Geometry: see drawing. Coordinates: mm, zero at the bounding-box minimum. A direction names the side the tool comes from. Give positions to 0.01 mm unless a question says otherwise; leave off trailing zeros. Write each loop counter-clockwise with the first axis right and the second up, starting at its lowest first coordinate (ties: lowest second). Pieces come first, ordered by that corner, then holes. Notation, with made-up numbers: (41.25, 77) -> (64.25, 77) arc R6 cw to (64.25, 84) -> close; hole circle Ø10 at (-22, -2). An arc over 180 degrees is marked (long way). Use one line per item in the form item = value. Start each with the question number.
(1) Cut plane D-D, the plane z = 40.5. Output: boundary loops of the cut face in (x, y).
(2) Cut plane A-A, the plane y = 29.2. Output: boundary loops of the cut face in (x, z), and give its area (3 significant figures).
(3) Cut plane C-C, the plane y = 9.2. Output: boundary loops of the cut face in (x, z).
(4) First-contact query: P1, Ø8, axis at y = 17.5, z = 39.5, coming from the +X side; P2, Ø5, axis at x = 21, z = 29, coming from the +Y side; P3, Ø6.5, axis at x = 6, y = 29.2, coming from the -Z side; P4, Ø4, axis at x = 6, y = 9.2, coming from the -Z side. Flat tips, straight axial feed; report the tip coordinate or a pass-through.
(5) Set-up query: the marked faces 1, 2 and 3. Return all of +Z, -Z, +X, -X, +Y, -Y with unobstructed straight access to the full face (end or side cutting, diameter ignored); none if empty.
(6) Cut plane B-B, the plane x = 6. Output: boundary loops of the cut face in (y, z), and give its area (4 significant figures).
(7) Draft query along Z for the marked faces 4, 5 and 6. Return one class per face: pulls with the +Z half, pulls with the -Z half, needs draft (parallel to the pull), parting line crosses it, or undercut.
(8) Material intervals for line 1 along X through (y, z) = (9, 70); line 2 along Y through (x, z) = (6, 70.5); line 3 along X through (y, z) = (7, 8), sorted ascending. Write a range as from..to.
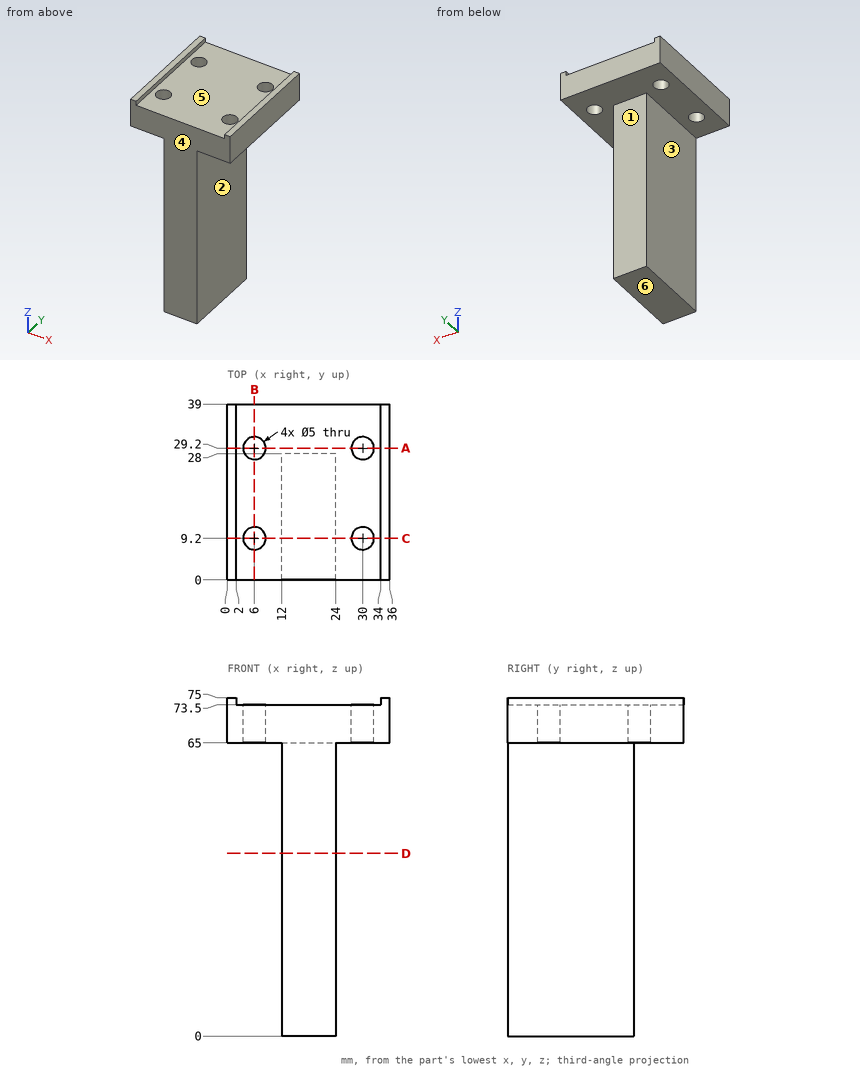
Geometry says:
q1.outline = (12, 0) -> (24, 0) -> (24, 28) -> (12, 28) -> close
q2.outline = (0, 65) -> (3.5, 65) -> (3.5, 73.5) -> (2, 73.5) -> (2, 75) -> (0, 75) -> close; (8.5, 65) -> (27.5, 65) -> (27.5, 73.5) -> (8.5, 73.5) -> close; (32.5, 65) -> (36, 65) -> (36, 75) -> (34, 75) -> (34, 73.5) -> (32.5, 73.5) -> close
q2.area = 227 mm^2
q3.outline = (0, 65) -> (3.5, 65) -> (3.5, 73.5) -> (2, 73.5) -> (2, 75) -> (0, 75) -> close; (8.5, 65) -> (12, 65) -> (12, 0) -> (24, 0) -> (24, 65) -> (27.5, 65) -> (27.5, 73.5) -> (8.5, 73.5) -> close; (32.5, 65) -> (36, 65) -> (36, 75) -> (34, 75) -> (34, 73.5) -> (32.5, 73.5) -> close
q4.P1 = 24
q4.P2 = 28
q4.P3 = 65
q4.P4 = through
q5.face_1 = -Z, +X, -X, +Y
q5.face_2 = -Z, +X, +Y, -Y
q5.face_3 = -Z, -X, +Y, -Y
q6.outline = (0, 65) -> (6.7, 65) -> (6.7, 73.5) -> (0, 73.5) -> close; (11.7, 65) -> (26.7, 65) -> (26.7, 73.5) -> (11.7, 73.5) -> close; (31.7, 65) -> (39, 65) -> (39, 73.5) -> (31.7, 73.5) -> close
q6.area = 246.5 mm^2
q7.face_4 = needs draft
q7.face_5 = pulls with the +Z half
q7.face_6 = pulls with the -Z half
q8.line_1 = 0..3.51, 8.49..27.51, 32.49..36
q8.line_2 = 0..6.7, 11.7..26.7, 31.7..39
q8.line_3 = 12..24
